```python
from build123d import *

# Parameters (mm, degrees)
SKETCH_1_R             = 35
EXTRUDE_1_DEPTH        = 15
CUT_EXTRUDE_1_DEPTH    = 15
FILLET_1_R             = 3
FILLET_1_OF_MIRROR_1_R = 3
SKETCH_3_R             = 17
SKETCH_3_R_2           = 13.5
CUT_EXTRUDE_2_DEPTH    = 3.5
CUT_EXTRUDE_3_DEPTH    = 4
SKETCH_5_R             = 8
CUT_EXTRUDE_4_DEPTH    = 50.21908641
SKETCH_6_R             = 2.25
CUT_EXTRUDE_5_DEPTH    = 50.21908641
CHAMFER_1_SIZE         = 1


with BuildPart() as part:
    # 草图1 → 凸台-拉伸1 (new body)
    with BuildSketch(Plane.XY):
        Circle(SKETCH_1_R)
    extrude(amount=EXTRUDE_1_DEPTH)

    # 草图2 → 切除-拉伸1 (cut)
    with BuildSketch(Plane.XY.offset(15)):
        with BuildLine():
            Line((-16.670675913, 32.718043682), (-10.214786244, 20.047646794))
            ThreePointArc((-10.214786244, 20.047646794), (0, 22.5), (10.214786244, 20.047646794))
            Line((10.214786244, 20.047646794), (16.670675913, 32.718043682))
            ThreePointArc((16.670675913, 32.718043682), (0, 36.720318868), (-16.670675913, 32.718043682))
        make_face()
    cut_extrude_1 = extrude(amount=-CUT_EXTRUDE_1_DEPTH, mode=Mode.SUBTRACT)

    # 圆角1
    fillet_1_edges = [part.edges().sort_by_distance(p)[0] for p in [
        (-10.214786244, 20.047646794, 7.5),
        (10.214786244, 20.047646794, 7.5),
    ]]
    fillet(fillet_1_edges, radius=FILLET_1_R)

    # 镜向1: 切除-拉伸1 across plane
    add(cut_extrude_1.mirror(Plane.ZX), mode=Mode.SUBTRACT)

    # 圆角1 of 镜向1
    fillet_1_of_mirror_1_edges = [part.edges().sort_by_distance(p)[0] for p in [
        (-10.214786244, -20.047646794, 7.5),
        (10.214786244, -20.047646794, 7.5),
    ]]
    fillet(fillet_1_of_mirror_1_edges, radius=FILLET_1_OF_MIRROR_1_R)

    # 草图3 → 切除-拉伸2 (cut)
    with BuildSketch(Plane.XY.offset(15)):
        Circle(SKETCH_3_R)
        Circle(SKETCH_3_R_2, mode=Mode.SUBTRACT)
    extrude(amount=-CUT_EXTRUDE_2_DEPTH, mode=Mode.SUBTRACT)

    # 草图4 → 切除-拉伸3 (cut)
    with BuildSketch(Plane.XY.offset(15)):
        with BuildLine():
            ThreePointArc((21.110164899, 7.785302689), (22.5, 0), (21.110164899, -7.785302689))
            ThreePointArc((21.110164899, -7.785302689), (24.781668408, -11.69838536), (25.712111329, -6.413839024))
            ThreePointArc((25.712111329, -6.413839024), (26.5, 0), (25.712111329, 6.413839024))
            ThreePointArc((25.712111329, 6.413839024), (24.781668408, 11.69838536), (21.110164899, 7.785302689))
        make_face()
    cut_extrude_3 = extrude(amount=-CUT_EXTRUDE_3_DEPTH, mode=Mode.SUBTRACT)

    # 镜向2: 切除-拉伸3 across plane
    add(cut_extrude_3.mirror(Plane(origin=(0, 0, 0), x_dir=(0, 0, 1), z_dir=(1, 0, 0))), mode=Mode.SUBTRACT)

    # 草图5 → 切除-拉伸4 (cut, through all)
    with BuildSketch(Plane.XY.offset(15)):
        Circle(SKETCH_5_R)
    extrude(amount=-CUT_EXTRUDE_4_DEPTH, mode=Mode.SUBTRACT)

    # 草图6 → 切除-拉伸5 (cut, through all)
    with BuildSketch(Plane.XY.offset(15)):
        with Locations((-31, 0)):
            Circle(SKETCH_6_R)
        with Locations((31, 0)):
            Circle(SKETCH_6_R)
    extrude(amount=-CUT_EXTRUDE_5_DEPTH, mode=Mode.SUBTRACT)

    # 倒角1
    chamfer_1_edges = [part.edges().sort_by_distance(p)[0] for p in [
        (35, 0, 15),
        (-35, 0, 15),
    ]]
    chamfer(chamfer_1_edges, length=CHAMFER_1_SIZE)


solid = part.part
```
For this review, take the finished solid that the model builds, in its own axes (mm). A direction names the side the tool comes from. Give positions to 0.01 mm unless a question says otherwise; leave off trailing zeros. Write each loop counter-clockwise with the first axis right and the second up, starting at its lowest first coordinate (ties: lowest second). Pieces come first, ordered by that corner, then holes.
Item 1: Take a section at A-A (x = 0). Give the boundary of the cut face in (y, z).
Item 2: Machinability: for faces 5 (the face through (9.945, -21.143, 7.395)), 6 (the face through (-24.87, 11.67, 13.03)), which of the approach directions +Z, -Z, +X, -X, +Y, -Y give a long, thin tool a straight path to every point of the face, cutting with its end or side? Answer none if there is none.
Item 3: Take a section at C-C (z = 5.25). Give the boundary of the cut face in (x, y).
Item 4: Insertion check: P1, Ø5, axis at x = 23.92, y = -8.82, coming from the +Z side; P2, Ø2.5, axis at x = -31, y = 0, coming from the +Z side (1 decimal); P3, Ø5, axis at y = 19, z = 12.5, coming from the +X side; P4, Ø4, axis at x = -1.5, z = 12, coming from the +Y side. Each pin has a flat end and moves straight along its axis. Give the tip position at first contact, or say it passes through.
Item 5: Take a section at B-B (y = 0). Give the number of separate pieces and of enclosed holes in the cut face, and give its area (4 significant figures).
Item 6: Wall thickness on probe 1 along X at (y, z) = (-12.5, 13.5); probe 2 along Y at (x, z) = (8.5, 1.25); probe 3 along Y at (x, z) = (6.5, 13.75): over which ranges is each line inside the solid? List them lowest first.
Item 7: The part is to be moulded in two halves that separate along X. For faces 1 (the face through (-24.692, -11.724, 13.028)), 2 (the face through (34.17, 0.526, 14.826)), 3 (the face through (24.692, -11.724, 13.028)), 4 (the face through (-8.3, 0.4, 0)), say which applies: +X half, -X half, draft (parallel to the pull), parting line (faces both ways), or undercut.
Established:
1. outline: (-22.5, 0) - (-8, 0) - (-8, 15) - (-13.5, 15) - (-13.5, 11.5) - (-17, 11.5) - (-17, 15) - (-22.5, 15) - close; (8, 0) - (22.5, 0) - (22.5, 15) - (17, 15) - (17, 11.5) - (13.5, 11.5) - (13.5, 15) - (8, 15) - close
2. face 5: +Z, -Z, -Y
2. face 6: +Z
3. outline: (-15.89, -31.19) - (-11.5, -22.56) arc R3 cw to (-7.79, -21.11) arc R22.5 ccw to (7.79, -21.11) arc R3 cw to (11.5, -22.56) - (15.89, -31.19) arc R35 ccw to (15.89, 31.19) - (11.5, 22.56) arc R3 cw to (7.79, 21.11) arc R22.5 ccw to (-7.79, 21.11) arc R3 cw to (-11.5, 22.56) - (-15.89, 31.19) arc R35 ccw to start; hole circle Ø4.5 at (-31, 0); hole circle Ø16 at (0, 0); hole circle Ø4.5 at (31, 0)
4. P1: stops at z = 11
4. P2: passes through
4. P3: stops at x = 30.87
4. P4: stops at y = 22.5
5. separate pieces: 4
5. enclosed holes: 0
5. area: 617.5 mm2
6. probe 1: x = -32.69 to -11.52, -5.1 to 5.1, 11.52 to 32.69
6. probe 2: y = -20.94 to 20.94
6. probe 3: y = -21.54 to -15.71, -11.83 to -4.66, 4.66 to 11.83, 15.71 to 21.54
7. face 1: undercut
7. face 2: +X half
7. face 3: undercut
7. face 4: draft
